Build history of the part. All positions in model axes, mm. Coordinates: 2 decimals unless noted, no trailing zeros. Loops run counter-clockwise (first coordinate to the right, second up) from the corner with the lowest first, then second, coordinate; pieces in that order, holes last.
Item 1: Drill centre lines: line 1 along X through (y, z) = (-37.5, 0.65); line 2 along Y through (x, z) = (375.5, 0.65). Where is each one in solid material? Low to high.
Item 2: Cut at C-C (z = 0.5). List the corners of the cut face in (x, y).
Item 3: Cut at B-B (y = 30). List the corners of the cut face in (x, z), and give its area (3 significant figures).
Item 4: Cut at A-A (x = 201.5). List the corners of the cut face in (y, z).
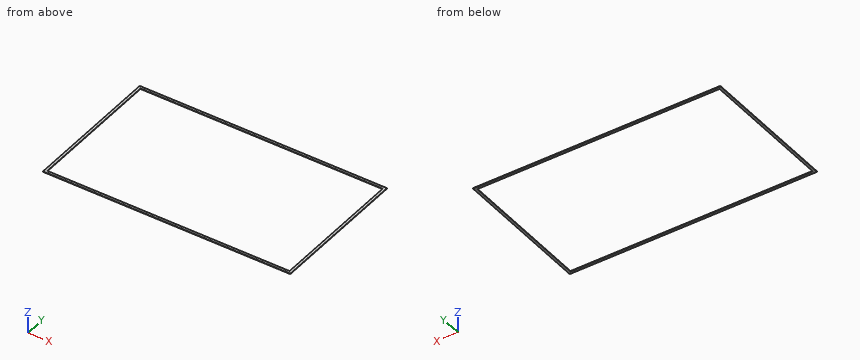
from build123d import *

# Parameters (mm, degrees)
SKETCH_1_W      = 974.6
SKETCH_1_H      = 557
SKETCH_1_W_2    = 954.6
SKETCH_1_H_2    = 537
EXTRUDE_1_DEPTH = 2
FILLET_1_R      = 0.2


with BuildPart() as part:
    # 草图1 → 凸台-拉伸1 (new body)
    with BuildSketch(Plane.XY):
        Rectangle(SKETCH_1_W, SKETCH_1_H)
        Rectangle(SKETCH_1_W_2, SKETCH_1_H_2, mode=Mode.SUBTRACT)
    extrude(amount=EXTRUDE_1_DEPTH)

    # 圆角1
    fillet_1_edges = [part.edges().sort_by_distance(p)[0] for p in [
        (477.3, -268.5, 1),
        (477.3, 268.5, 1),
        (-477.3, 268.5, 1),
        (-477.3, -268.5, 1),
    ]]
    fillet(fillet_1_edges, radius=FILLET_1_R)


solid = part.part
Filled sheet:
1. line 1: x = -487.3 to -477.3, 477.3 to 487.3
1. line 2: y = -278.5 to -268.5, 268.5 to 278.5
2. outline: (-487.3, -278.5) - (487.3, -278.5) - (487.3, 278.5) - (-487.3, 278.5) - close; hole (-477.3, -268.3) arc R0.2 ccw to (-477.1, -268.5) - (477.1, -268.5) arc R0.2 ccw to (477.3, -268.3) - (477.3, 268.3) arc R0.2 ccw to (477.1, 268.5) - (-477.1, 268.5) arc R0.2 ccw to (-477.3, 268.3) - close
3. outline: (-487.3, 0) - (-477.3, 0) - (-477.3, 2) - (-487.3, 2) - close; (477.3, 0) - (487.3, 0) - (487.3, 2) - (477.3, 2) - close
3. area: 40.0 mm2
4. outline: (-278.5, 0) - (-268.5, 0) - (-268.5, 2) - (-278.5, 2) - close; (268.5, 0) - (278.5, 0) - (278.5, 2) - (268.5, 2) - close
